from build123d import *

# Parameters (mm, degrees)
SKETCH1_R           = 7
BOSS_EXTRUDE1_DEPTH = 6


with BuildPart() as part:
    # Sketch1 → Boss-Extrude1 (new body)
    with BuildSketch(Plane(origin=(0, 0, 0), x_dir=(1, 0, 0), z_dir=(0, 1, 0))):
        with BuildLine():
            Line((40, -20), (-50, -20))
            Line((-50, -20), (-50, 20))
            Line((-50, 20), (40, 20))
            ThreePointArc((40, 20), (47.071067812, 17.071067812), (50, 10))
            Line((50, 10), (50, -10))
            ThreePointArc((50, -10), (47.071067812, -17.071067812), (40, -20))
        make_face()
        with Locations(Location((25, 0, 0), (0, 0, 270))):
            Circle(SKETCH1_R, mode=Mode.SUBTRACT)
    extrude(amount=BOSS_EXTRUDE1_DEPTH)


solid = part.part
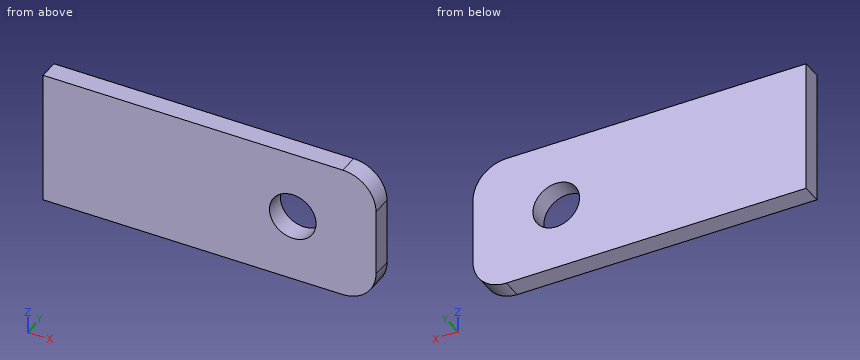
The model under review builds one solid part; all positions refer to its coordinate system, in mm. Round coordinates to 2 decimals unless told otherwise and drop trailing zeros. Write each loop counter-clockwise with the first axis right and the second up, starting at its lowest first coordinate (ties: lowest second). Pieces come first, ordered by that corner, then holes. Notation, with made-up numbers: (25.5, 17.5) -> (70.5, 17.5) arc R19 cw to (70.5, 47.5) -> close; hole circle Ø1 at (9.25, 39.25). An arc over 180 degrees is marked (long way). Answer as a JSON object with one key per item and string values.
1. We need section C-C on y = 1.1. State the section outline as (x, z) points.
Results found:
{"outline": "(-50, -20) -> (40, -20) arc R10 ccw to (50, -10) -> (50, 10) arc R10 ccw to (40, 20) -> (-50, 20) -> close; hole circle Ø14 at (25, 0)"}
2. We need section A-A on z = 0. State the section outline as (x, y) points, and give its area (3 significant figures).
Results found:
{"outline": "(-50, 0) -> (18, 0) -> (18, 6) -> (-50, 6) -> close; (32, 0) -> (50, 0) -> (50, 6) -> (32, 6) -> close", "area": "516 mm^2"}
3. To check wall thickness, follow line 1 along X through (y, z) = (3.65, 0); line 2 along X through (y, z) = (5.4, 2); line 3 along Z through (x, y) = (19, 2.85). State the ranges of each line that lie inside material, in increasing order.
Results found:
{"line 1": "x = -50 to 18, 32 to 50", "line 2": "x = -50 to 18.29, 31.71 to 50", "line 3": "z = -20 to -3.61, 3.61 to 20"}
4. We need section B-B on x = 25. State the section outline as (y, z) points.
Results found:
{"outline": "(0, -20) -> (6, -20) -> (6, -7) -> (0, -7) -> close; (0, 7) -> (6, 7) -> (6, 20) -> (0, 20) -> close"}
